from build123d import *

# Parameters (mm, degrees)
BASE_BLOCK_DEPTH                       = 45
SLOTTED_TAB_DEPTH                      = 8
ANGLED_LIP_DEPTH                       = 60
CLEVIS_SLOT_DEPTH                      = 9
CLEVIS_CROSS_HOLE_M14_15_D             = 15
COUNTERBORED_BOLT_HOLE_M10_D           = 12
COUNTERBORED_BOLT_HOLE_M10_DEPTH       = 21
COUNTERBORED_BOLT_HOLE_M10_CBORE_D     = 24
COUNTERBORED_BOLT_HOLE_M10_CBORE_DEPTH = 9


with BuildPart() as part:
    # Base Block Sketch → Base Block (new body)
    with BuildSketch(Plane(origin=(0, 0, 0), x_dir=(1, 0, 0), z_dir=(0, 1, 0))):
        with BuildLine():
            Line((-60, 30), (-60, 9))
            Line((-60, 9), (-12, 9))
            ThreePointArc((-12, 9), (15, 0), (-12, -9))
            Line((-12, -9), (-60, -9))
            Line((-60, -9), (-60, -30))
            Line((-60, -30), (0, -30))
            ThreePointArc((0, -30), (30, 0), (0, 30))
            Line((0, 30), (-60, 30))
        make_face()
    extrude(amount=BASE_BLOCK_DEPTH)

    # Slotted Tab Sketch → Slotted Tab (add)
    with BuildSketch(Plane(origin=(0, 18, 0), x_dir=(-1, 0, 0), z_dir=(0, -1, 0))):
        with BuildLine():
            Line((0, 30), (-51, 30))
            Line((-51, 30), (-90, 30))
            Line((-90, 30), (-90, -30))
            Line((-90, -30), (-69, -30))
            Line((-69, -30), (-69, 0))
            ThreePointArc((-69, 0), (-60, 9), (-51, 0))
            Line((-51, 0), (-51, -30))
            Line((-51, -30), (0, -30))
            ThreePointArc((0, -30), (-30, 0), (0, 30))
        make_face()
    extrude(amount=-SLOTTED_TAB_DEPTH)

    # Angled Lip Sketch → Angled Lip (add)
    with BuildSketch(Plane.XY.offset(30)):
        Polygon((90, 18), (137, 65), (133, 69), (90, 26), align=None)
    extrude(amount=-ANGLED_LIP_DEPTH)

    # Clevis Slot Sketch → Clevis Slot (cut)
    with BuildSketch(Plane(origin=(32, -32, 0), x_dir=(0, 0, 1), z_dir=(-0.7071067811865439, 0.7071067811865512, 0))):
        with BuildLine():
            Line((-14.311818372, 132.015695434), (-30, 82.024386618))
            Line((-30, 82.024386618), (-33.812783533, 82.024386618))
            Line((-33.812783533, 82.024386618), (-33.812783533, 155.319200691))
            Line((-33.812783533, 155.319200691), (36.02403622, 155.319200691))
            Line((36.02403622, 155.319200691), (36.02403622, 82.024386618))
            Line((36.02403622, 82.024386618), (30, 82.024386618))
            Line((30, 82.024386618), (14.311818372, 132.015695434))
            ThreePointArc((14.311818372, 132.015695434), (0, 142.524386618), (-14.311818372, 132.015695434))
        make_face()
    extrude(amount=-CLEVIS_SLOT_DEPTH, mode=Mode.SUBTRACT)

    # Clevis Cross Hole M14 Ø15 (through all)
    with Locations(Plane(origin=(32, -32, 0), x_dir=(0.7071067811865512, 0.7071067811865439, 0), z_dir=(-0.7071067811865439, 0.7071067811865512, 0))):
        with Locations((127.524386618, 0)):
            Hole(CLEVIS_CROSS_HOLE_M14_15_D / 2)

    # Counterbored Bolt Hole M10
    with Locations(Plane.XY.offset(30)):
        with Locations((-36, 22.5)):
            counterbored_bolt_hole_m10 = CounterBoreHole(COUNTERBORED_BOLT_HOLE_M10_D / 2, COUNTERBORED_BOLT_HOLE_M10_CBORE_D / 2, COUNTERBORED_BOLT_HOLE_M10_CBORE_DEPTH, depth=COUNTERBORED_BOLT_HOLE_M10_DEPTH)

    # Bolt Hole Mirror: Counterbored Bolt Hole M10 across plane
    add(counterbored_bolt_hole_m10.mirror(Plane.XY), mode=Mode.SUBTRACT)


solid = part.part
Can you work these out from the model? Positions are in its coordinate system, mm. A direction names the side the tool comes from. Round coordinates to 2 decimals unless told otherwise and drop trailing zeros. Order: outer loops, then holes, each group sorted by start corner. A loop starts at its lowest first (then second) coordinate and runs counter-clockwise, first axis right, second up. Notation, with made-up numbers: (18, 70) -> (25, 70) arc R29 ccw to (25, 101) -> close; hole circle Ø2 at (75.5, -24). An arc over 180 degrees is marked (long way). Write each question's results on one line, items separated by ' | '. Start each with the question number.
Item 1: If we section it at B-B, the plane z = 26: Write out the boundary of the cut face in (x, y).
Item 2: If we section it at A-A, the plane x = -36: Write out the boundary of the cut face in (y, z), then the cut area to 3 significant figures.
Item 3: Will these pins go through, and if not, where does the flat tip stop? pin 1 (18 mm diameter, centred on x = 65.5, z = 2, fed in from -Y); pin 2 (15.5 mm diameter, centred on x = -36, y = 22.5, fed in from +Z); pin 3 (3 mm diameter, centred on y = 34, z = 2.5, fed in from +X).
Item 4: Please list where these lines run through material, in increasing order: L1, parallel to Z at x = -25, y = 31; L2, parallel to Y at x = -36, z = 13.75; L3, parallel to X at y = 28, z = 10.
Item 5: Which directions (+Z, -Z, +X, -X, +Y, -Y) give clear straight access to the entire face, cutting with the end or side of a thin tool? Please do faces 5 (the cylindrical face through (29.993, 8.874, 0.66)), 6 (the flat face through (-42, 20, 21)), 7 (the flat face through (51, 22, 15)).
Item 6: If we section it at D-D, the plane y = 37: Write out the boundary of the cut face in (x, z).
Item 7: If we section it at C-C, the plane y = 8: Write out the boundary of the cut face in (x, z), then the cut area to 3 significant figures.
Item 8: Thinking about a two-plate mould opening in X: for faces 1 (the cylindrical face through (29.993, 35.367, 0.66)), 2 (the flat face through (-31, 17, -9)), 3 (the flat face through (108, 36, 0)), 4 (the flat face through (-60, 22, 19)), which applies, +X half, -X half, draft (parallel to the pull), parting line (faces both ways), or undercut?
Results:
1) outline: (-60, 0) -> (14.97, 0) -> (14.97, 18) -> (51, 18) -> (51, 26) -> (14.97, 26) -> (14.97, 45) -> (-60, 45) -> close; (69, 18) -> (90, 18) -> (103.01, 31.01) -> (99.01, 35.01) -> (90, 26) -> (69, 26) -> close; hole circle Ø24 at (-36, 22.5)
2) outline: (0, -30) -> (10.5, -30) -> (10.5, -21) -> (16.5, -21) -> (16.5, -9) -> (0, -9) -> close; (0, 9) -> (16.5, 9) -> (16.5, 21) -> (10.5, 21) -> (10.5, 30) -> (0, 30) -> close; (28.5, -21) -> (34.5, -21) -> (34.5, -30) -> (45, -30) -> (45, -9) -> (28.5, -9) -> close; (28.5, 9) -> (45, 9) -> (45, 30) -> (34.5, 30) -> (34.5, 21) -> (28.5, 21) -> close | area: 1,170 mm2
3) pin 1: stops at y = 18 | pin 2: stops at z = 21 | pin 3: stops at x = 107.5
4) L1: z = -30 to -9, 9 to 30 | L2: y = 0 to 16.5, 28.5 to 45 | L3: x = -60 to -38.4, -33.6 to -11.18, 11.18 to 28.28, 92 to 100
5) face 5: +X, -Y | face 6: +Z | face 7: +Z, +Y, -Y
6) outline: (-60, -30) -> (0, -30) arc R30 ccw to (0, 30) -> (-60, 30) -> (-60, 9) -> (-12, 9) arc R15 cw (long way) to (-12, -9) -> (-60, -9) -> close; (101, -25.12) -> (109, -23.34) -> (109, 23.34) -> (101, 25.12) -> close
7) outline: (-60, -30) -> (0, -30) arc R30 ccw to (0, 30) -> (-60, 30) -> (-60, 9) -> (-12, 9) arc R15 cw (long way) to (-12, -9) -> (-60, -9) -> close | area: 3,480 mm2
8) face 1: undercut | face 2: draft | face 3: +X half | face 4: -X half
